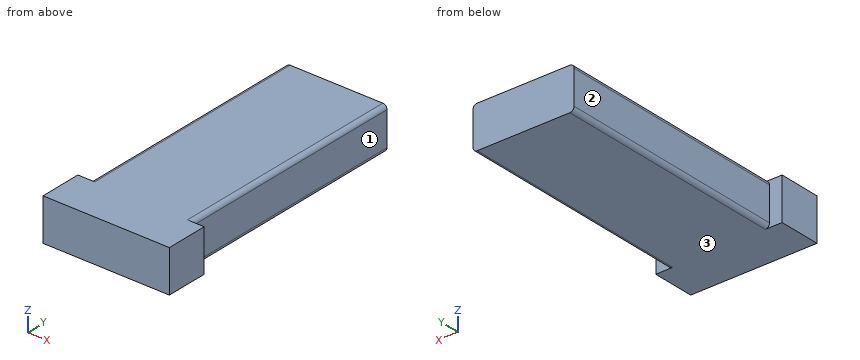
```python
from build123d import *

# Parameters (mm, degrees)
SKETCH1_W           = 15
SKETCH1_H           = 5
BOSS_EXTRUDE1_DEPTH = 2.5
SKETCH3_W           = 12
SKETCH3_H           = 5
BOSS_EXTRUDE2_DEPTH = 28
FILLET1_R           = 0.5


with BuildPart() as part:
    # Sketch1 → Boss-Extrude1 (new, symmetric)
    with BuildSketch(Plane.XY):
        with Locations((0, -52.27)):
            Rectangle(SKETCH1_W, SKETCH1_H)
    extrude(amount=BOSS_EXTRUDE1_DEPTH, both=True)

    # Sketch3 → Boss-Extrude2 (add)
    with BuildSketch(Plane(origin=(0, -49.77, 0), x_dir=(1, 0, 0), z_dir=(0, 1, 0))):
        Rectangle(SKETCH3_W, SKETCH3_H)
    extrude(amount=BOSS_EXTRUDE2_DEPTH)

    # Fillet1
    fillet1_edges = [part.edges().sort_by_distance(p)[0] for p in [
        (-6, -35.77, -2.5),
        (-6, -35.77, 2.5),
        (6, -35.77, 2.5),
        (6, -35.77, -2.5),
    ]]
    fillet(fillet1_edges, radius=FILLET1_R)


solid = part.part
```
For this review, take the finished solid that the model builds, in its own axes (mm). Face numbers are marked on the shaded views. A direction names the side the tool comes from. Round coordinates to 2 decimals unless told otherwise and drop trailing zeros. Write each loop counter-clockwise with the first axis right and the second up, starting at its lowest first coordinate (ties: lowest second). Pieces come first, ordered by that corner, then holes.
1) Machinability: for the marked faces 1, 2 and 3, which of the approach directions +Z, -Z, +X, -X, +Y, -Y give a long, thin tool a straight path to every point of the face, cutting with its end or side? Answer none if there is none.
Answer below:
face 1: +Z, -Z, +X, +Y
face 2: +Z, -Z, -X, +Y
face 3: -Z, +X, -X, +Y, -Y
2) Take a section at A-A on y = -37. Give the boundary of the cut face in (x, z), then the cut area to 3 significant figures.
Answer below:
outline: (-6, -2) arc R0.5 ccw to (-5.5, -2.5) - (5.5, -2.5) arc R0.5 ccw to (6, -2) - (6, 2) arc R0.5 ccw to (5.5, 2.5) - (-5.5, 2.5) arc R0.5 ccw to (-6, 2) - close
area: 59.8 mm2
3) For line 1 along X through (y, z) = (-25.5, -2); line 2 along X through (y, z) = (-39, -2.25), list the stretches that pass through material, from the lowest coordinate up.
Answer below:
line 1: x = -6 to 6
line 2: x = -5.93 to 5.93
4) Take a section at B-B on z = -1. Give the boundary of the cut face in (x, y), then the cut area to 3 significant figures.
Answer below:
outline: (-7.5, -54.77) - (7.5, -54.77) - (7.5, -49.77) - (6, -49.77) - (6, -21.77) - (-6, -21.77) - (-6, -49.77) - (-7.5, -49.77) - close
area: 411 mm2
5) Insertion check: pin 1 Ø3 at (y, z) = (-29, 0.5) entering from -X; pin 2 Ø1.6 at (x, z) = (-7, 0) entering from +Y; pin 3 Ø2 at (y, z) = (-42.5, 0) entering from +X. Each pin has a flat end and moves straight along its axis. Give the tip position at first contact, or say it passes through.
Answer below:
pin 1: stops at x = -6
pin 2: stops at y = -49.77
pin 3: stops at x = 6
